Input: dimensioned drawing with shaded views. Units: mm. Origin: part minimum x, y, z. A direction names the side the tool comes from. Round coordinates to 2 decimals unless told otherwise and drop trailing zeros. Loops run counter-clockwise (first coordinate to the right, second up) from the corner with the lowest first, then second, coordinate; pieces in that order, holes last. Notation, with made-up numbers: M 41,40.5 L 86,40.5 A21 ccw 86,50.5 Z; hole C 51.25,-4 d3. An arc over 180 degrees is marked long. One line per item, written item: value.
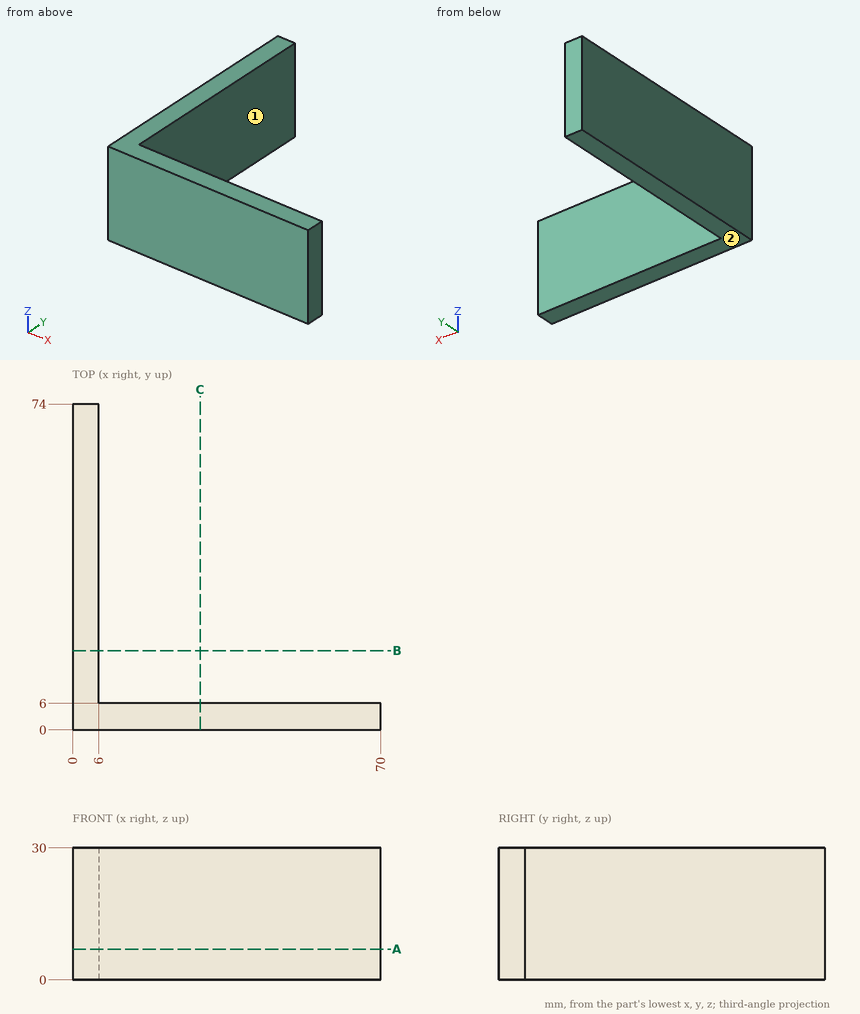
1. Pin query (flat end, axial travel): pin 1 (6 mm diameter, centred on y = 35.5, z = 21, fed in from +X); pin 2 (9 mm diameter, centred on x = 42, z = 14.5, fed in from +Y). Return the tip coordinate at first contact, or that it passes through.
Report:
pin 1: stops at x = 6
pin 2: stops at y = 6
2. Ray query, line 1 (X direction, y = 33, z = 9.25). Return the intervals inside material, ascending. Write a range as [from, to].
Report:
line 1: x = [0, 6]
3. Reachability of the marked faces 1 and 2 from +Z, -Z, +X, -X, +Y, -Y: full face, straight path, thin tool, end or side. Return the list, or none.
Report:
face 1: +Z, -Z, +X, +Y
face 2: -Z, +X, -X, +Y, -Y
4. Section query B-B (y = 18). Return the cut outline in (x, z), and give its area (3 significant figures).
Report:
outline: M 0,0 L 6,0 L 6,30 L 0,30 Z
area: 180 mm2
5. Section query A-A (z = 7). Return the cut outline in (x, y).
Report:
outline: M 0,0 L 70,0 L 70,6 L 6,6 L 6,74 L 0,74 Z
